```python
from build123d import *

# Parameters (mm, degrees)
HOUSING_BASE_PROFILE_SKETCH_R  = 52.5
HOUSING_CYLINDER_DEPTH         = 63
MOUNTING_FLANGE_DEPTH          = 12
SKETCH1_4_R                    = 12
LUG_BOSSES_DEPTH               = 25
BORE_AND_LUG_HOLES_SKETCH_R    = 6
BORE_AND_LUG_HOLES_SKETCH_R_2  = 46.5
BORE_AND_LUG_HOLES_2X_12_DEPTH = 129.939908485
FLANGE_RELIEF_POCKETS_DEPTH    = 3


with BuildPart() as part:
    # Housing Base Profile Sketch → Housing Cylinder (new body)
    with BuildSketch(Plane(origin=(0, 0, 0), x_dir=(1, 0, 0), z_dir=(0, 1, 0))):
        with Locations(Location((0, 0, 0), (0, 0, 270))):
            Circle(HOUSING_BASE_PROFILE_SKETCH_R)
    extrude(amount=HOUSING_CYLINDER_DEPTH)

    # Sketch1_3 → Mounting Flange (add)
    with BuildSketch(Plane(origin=(0, 0, 0), x_dir=(1, 0, 0), z_dir=(0, 1, 0))):
        with BuildLine():
            Line((-24.3, 46.537726631), (-93.054285714, 10.637194659))
            ThreePointArc((-93.054285714, 10.637194659), (-81.281134692, 10.262831689), (-75.5, 0))
            ThreePointArc((-75.5, 0), (-81.281134692, -10.262831689), (-93.054285714, -10.637194659))
            Line((-93.054285714, -10.637194659), (-24.3, -46.537726631))
            ThreePointArc((-24.3, -46.537726631), (-52.5, 0), (-24.3, 46.537726631))
        make_face()
        with BuildLine():
            Line((93.054285714, 10.637194659), (24.3, 46.537726631))
            ThreePointArc((24.3, 46.537726631), (44.899888641, 27.207535721), (52.5, 0))
            ThreePointArc((52.5, 0), (45.157075755, -26.778508346), (25.182342504, -46.066252572))
            Line((25.182342504, -46.066252572), (87.5, -12))
            ThreePointArc((87.5, -12), (75.845680288, 2.859516051), (93.054285714, 10.637194659))
        make_face()
    extrude(amount=MOUNTING_FLANGE_DEPTH)

    # Sketch1_4 → Lug Bosses (add)
    with BuildSketch(Plane(origin=(0, 0, 0), x_dir=(1, 0, 0), z_dir=(0, 1, 0))):
        with Locations(Location((87.5, 0, 0), (0, 0, 270))):
            Circle(SKETCH1_4_R)
        with Locations(Location((-87.5, 0, 0), (0, 0, 117.57162794))):
            Circle(SKETCH1_4_R)
    extrude(amount=LUG_BOSSES_DEPTH)

    # Bore and Lug Holes Sketch → Bore and Lug Holes 2x_12 (cut, through all)
    with BuildSketch(Plane(origin=(0, 63, 0), x_dir=(1, 0, 0), z_dir=(0, 1, 0))):
        with Locations(Location((-87.5, 0, 0), (0, 0, 270))):
            Circle(BORE_AND_LUG_HOLES_SKETCH_R)
        with Locations(Location((0, 0, 0), (0, 0, 270))):
            Circle(BORE_AND_LUG_HOLES_SKETCH_R_2)
        with Locations(Location((87.5, 0, 0), (0, 0, 270))):
            Circle(BORE_AND_LUG_HOLES_SKETCH_R)
    extrude(amount=-BORE_AND_LUG_HOLES_2X_12_DEPTH, mode=Mode.SUBTRACT)

    # Flange Pockets Sketch → Flange Relief Pockets (cut)
    with BuildSketch(Plane(origin=(0, 12, 0), x_dir=(1, 0, 0), z_dir=(0, 1, 0))):
        with BuildLine():
            Line((-60.67046514, 20.916189471), (-72.83224793, 15.355373632))
            ThreePointArc((-72.83224793, 15.355373632), (-74.521451253, 13.240091694), (-73.819589316, 10.625667214))
            ThreePointArc((-73.819589316, 10.625667214), (-69.591109503, -0.257419194), (-73.582978557, -11.22950162))
            ThreePointArc((-73.582978557, -11.22950162), (-74.226651592, -13.864622877), (-72.481931561, -15.941671512))
            Line((-72.481931561, -15.941671512), (-60.177135194, -21.187902521))
            ThreePointArc((-60.177135194, -21.187902521), (-56.993480479, -20.657990086), (-56.132769828, -17.547420732))
            ThreePointArc((-56.132769828, -17.547420732), (-58.852375063, -0.116051975), (-56.53564235, 17.373419684))
            ThreePointArc((-56.53564235, 17.373419684), (-57.471032791, 20.466004181), (-60.67046514, 20.916189471))
        make_face()
        with BuildLine():
            Line((60.67046514, 20.916189471), (72.83224793, 15.355373632))
            ThreePointArc((72.83224793, 15.355373632), (74.521451253, 13.240091694), (73.819589316, 10.625667214))
            ThreePointArc((73.819589316, 10.625667214), (69.591109503, -0.257419194), (73.582978557, -11.22950162))
            ThreePointArc((73.582978557, -11.22950162), (74.226651592, -13.864622877), (72.481931561, -15.941671512))
            Line((72.481931561, -15.941671512), (60.177135194, -21.187902521))
            ThreePointArc((60.177135194, -21.187902521), (56.993480479, -20.657990086), (56.132769828, -17.547420732))
            ThreePointArc((56.132769828, -17.547420732), (58.852375063, -0.116051975), (56.53564235, 17.373419684))
            ThreePointArc((56.53564235, 17.373419684), (57.471032791, 20.466004181), (60.67046514, 20.916189471))
        make_face()
    extrude(amount=-FLANGE_RELIEF_POCKETS_DEPTH, mode=Mode.SUBTRACT)


solid = part.part
```
Model file for the job. Use its own axes, mm. A direction names the side the tool comes from. Give positions to 0.01 mm unless a question says otherwise; leave off trailing zeros. Loops run counter-clockwise (first coordinate to the right, second up) from the corner with the lowest first, then second, coordinate; pieces in that order, holes last. Notation, with made-up numbers: (47, -9) -> (93, -9) arc R20 ccw to (93, 28) -> close; hole circle Ø2 at (87, 85). An arc over 180 degrees is marked (long way). Write each question's results on one line, items separated by ' | '.
(1) Cut at A-A on x = 0. List the corners of the cut face in (y, z), and give its area (3 significant figures).
Geometry results:
outline: (0, -52.5) -> (63, -52.5) -> (63, -46.5) -> (0, -46.5) -> close; (0, 46.5) -> (63, 46.5) -> (63, 52.5) -> (0, 52.5) -> close | area: 756 mm²
(2) Cut at D-D on x = -87.5. List the corners of the cut face in (y, z).
Geometry results:
outline: (0, -13.54) -> (12, -13.54) -> (12, -12) -> (25, -12) -> (25, -6) -> (0, -6) -> close; (0, 6) -> (25, 6) -> (25, 12) -> (12, 12) -> (12, 13.54) -> (0, 13.54) -> close
(3) Pull direction X, two halves, no side cores. Call faces 1 (the flat face through (-56, 12, 0)), 2 (the flat face through (85, 25, -6)), 3 (the flat face through (-58.196, 5.916, -28.839)): released by +X, released by -X, zero draft, split by the parting line, or undercut.
Geometry results:
face 1: undercut | face 2: zero draft | face 3: released by -X
(4) Cut at B-B on z = -8.5. List the corners of the cut face in (x, y), and give its area (3 significant figures).
Geometry results:
outline: (-95.97, 0) -> (-45.72, 0) -> (-45.72, 63) -> (-51.81, 63) -> (-51.81, 12) -> (-58.35, 12) -> (-58.35, 9) -> (-72.2, 9) -> (-72.2, 12) -> (-79.03, 12) -> (-79.03, 25) -> (-95.97, 25) -> close; (45.72, 0) -> (95.97, 0) -> (95.97, 25) -> (79.03, 25) -> (79.03, 12) -> (72.2, 12) -> (72.2, 9) -> (58.35, 9) -> (58.35, 12) -> (51.81, 12) -> (51.81, 63) -> (45.72, 63) -> close | area: 2,180 mm²
(5) Probe line 1 along X through (y, z) = (6.75, 0); line 2 along X through (y, z) = (14, 0); line 3 along Z through (x, y) = (-1, 17). List the from-to ranges inside material, lowest first.
Geometry results:
line 1: x = -99.5 to -93.5, -81.5 to -46.5, 46.5 to 81.5, 93.5 to 99.5 | line 2: x = -99.5 to -93.5, -81.5 to -75.5, -52.5 to -46.5, 46.5 to 52.5, 75.5 to 81.5, 93.5 to 99.5 | line 3: z = -52.49 to -46.49, 46.49 to 52.49
(6) Tool access for faces 4 (the flat face through (-66.416, 10.521, 18.528)), 5 (the flat face through (-94, 25, 0)), 6 (the flat face through (-35, 63, -31)): list every direction of +Z, -Z, +X, -X, +Y, -Y with a clear straight run to the whole face (end or side of a thin tool).
Geometry results:
face 4: +Y | face 5: +Z, -Z, -X, +Y | face 6: +Z, -Z, +X, -X, +Y
(7) Cut at C-C on y = 54. List the corners of the cut face in (x, z), and give its area (3 significant figures).
Geometry results:
outline: circle Ø105 at (0, 0); hole circle Ø93 at (0, 0) | area: 1,870 mm²
(8) Flat gauge pins, fed straight in: pin 1 Ø20.5 at (x, z) = (69, -19.5) entering from +Y; pin 2 Ø14 at (x, z) = (87.5, 0) entering from +Y; pin 3 Ø12 at (x, y) = (-75, 9) entering from -Z. Where does each tip first touch, or does it go through?
Geometry results:
pin 1: stops at y = 12 | pin 2: stops at y = 25 | pin 3: stops at z = -23.2
